Work out the finished part from the listing and answer in its coordinate system (mm). A direction names the side the tool comes from. Coordinates: 2 decimals unless noted, no trailing zeros. Loops run counter-clockwise (first coordinate to the right, second up) from the corner with the lowest first, then second, coordinate; pieces in that order, holes last. Notation, with made-up numbers: (82, -2.5) - (102, -2.5) arc R19 cw to (102, 13.5) - close; hole circle Ø2 at (-15.5, 89). An arc over 180 degrees is marked (long way). Write each question's results on one line, items separated by ' | '. Start each with the question number.
1. Determine the mould class of faces 3 (the flat face through (35, 66, 8)), 4 (the cylindrical face through (2.85, 3.01, 3.94)), 5 (the flat face through (35, 20.5, 4)), 6 (the cylindrical face through (11.5, 14.9, 4.1)) for opening direction Y: released by +Y, released by -Y, zero draft, split by the parting line, or undercut.
2. A cutting plane is placed at C-C on y = 15. Determine the outline of the cut face in (x, z).
3. Find the intervals of material crossed by line 1 along Y through (x, z) = (43, 7.25); line 2 along X through (y, z) = (15, 3); line 3 along Y through (x, z) = (15, 1.25), in increasing order. Write a range as [from, to].
4. A cutting plane is placed at A-A on z = 1.5. Determine the outline of the cut face in (x, y).
5. This flat-tipped pin is pushed along its axis until it touches: P1, Ø1.5, axis at x = 7.5, z = 6, coming from the -Y side. Where does it stop, or does it pass through?
6. A cutting plane is placed at B-B on x = 46.5. Determine the outline of the cut face in (y, z), then the cut area to 3 significant figures.
7. Which of the six approach directions +Z, -Z, +X, -X, +Y, -Y give full straight-line access (tool end or side, diameter ignored) to faces 1 (the cylindrical face through (67.15, 126.99, 3.94)), 2 (the flat face through (35, 9.5, 4))?
from build123d import *

# Parameters (mm, degrees)
BOSS_EXTRUDE1_DEPTH = 8
CUT_EXTRUDE1_DEPTH  = 10


with BuildPart() as part:
    # Sketch1 → Boss-Extrude1 (new body)
    with BuildSketch(Plane.XY):
        with BuildLine():
            Line((10, 0), (60, 0))
            ThreePointArc((60, 0), (67.071067812, 2.928932188), (70, 10))
            Line((70, 10), (70, 120))
            ThreePointArc((70, 120), (67.071067812, 127.071067812), (60, 130))
            Line((60, 130), (10, 130))
            ThreePointArc((10, 130), (2.928932188, 127.071067812), (0, 120))
            Line((0, 120), (0, 10))
            ThreePointArc((0, 10), (2.928932188, 2.928932188), (10, 0))
        make_face()
    extrude(amount=BOSS_EXTRUDE1_DEPTH)

    # Sketch2 → Cut-Extrude1 (cut)
    with BuildSketch(Plane.XY.offset(8)):
        with BuildLine():
            Line((17, 20.5), (53, 20.5))
            ThreePointArc((53, 20.5), (58.5, 15), (53, 9.5))
            Line((53, 9.5), (17, 9.5))
            ThreePointArc((17, 9.5), (11.5, 15), (17, 20.5))
        make_face()
    extrude(amount=-CUT_EXTRUDE1_DEPTH, mode=Mode.SUBTRACT)


solid = part.part
Values:
1) face 3: zero draft | face 4: released by -Y | face 5: undercut | face 6: undercut
2) outline: (0, 0) - (11.5, 0) - (11.5, 8) - (0, 8) - close; (58.5, 0) - (70, 0) - (70, 8) - (58.5, 8) - close
3) line 1: [0, 9.5], [20.5, 130] | line 2: [0, 11.5], [58.5, 70] | line 3: [0, 9.88], [20.12, 130]
4) outline: (0, 10) arc R10 ccw to (10, 0) - (60, 0) arc R10 ccw to (70, 10) - (70, 120) arc R10 ccw to (60, 130) - (10, 130) arc R10 ccw to (0, 120) - close; hole (17, 9.5) - (53, 9.5) arc R5.5 ccw to (53, 20.5) - (17, 20.5) arc R5.5 ccw to start
5) P1: y = 0.15
6) outline: (0, 0) - (9.5, 0) - (9.5, 8) - (0, 8) - close; (20.5, 0) - (130, 0) - (130, 8) - (20.5, 8) - close | area: 952 mm^2
7) face 1: +Z, -Z, +X, +Y | face 2: +Z, -Z
